from build123d import *

# Parameters (mm, degrees)
SKETCH1_W           = 480
SKETCH1_H           = 600
BOSS_EXTRUDE1_DEPTH = 40
SKETCH4_W           = 120
SKETCH4_H           = 440
CUT_EXTRUDE3_DEPTH  = 387.264158317
FILLET1_R           = 20
M24_TAPPED_HOLE1_D  = 21


with BuildPart() as part:
    # Sketch1 → Boss-Extrude1 (new body)
    with BuildSketch(Plane(origin=(0, 0, 0), x_dir=(1, 0, 0), z_dir=(0, 1, 0))):
        Rectangle(SKETCH1_W, SKETCH1_H)
    extrude(amount=BOSS_EXTRUDE1_DEPTH)

    # Sketch4 → Cut-Extrude3 (cut, through all)
    with BuildSketch(Plane(origin=(0, 40, 0), x_dir=(1, 0, 0), z_dir=(0, 1, 0))):
        with Locations((-112, 0)):
            Rectangle(SKETCH4_W, SKETCH4_H)
    extrude(amount=-CUT_EXTRUDE3_DEPTH, mode=Mode.SUBTRACT)

    # Fillet1
    fillet1_edges = [part.edges().sort_by_distance(p)[0] for p in [
        (-52, 20, -220),
        (-52, 20, 220),
        (-172, 20, 220),
        (-172, 20, -220),
    ]]
    fillet(fillet1_edges, radius=FILLET1_R)

    # M24 Tapped Hole1 (through all)
    with Locations(Plane(origin=(0, 40, 0), x_dir=(1, 0, 0), z_dir=(0, 1, 0))):
        with Locations((-190, -270), (-190, 270), (190, 270), (190, -270), (190, 170), (190, -170)):
            Hole(M24_TAPPED_HOLE1_D / 2)


solid = part.part
Geometry: final body of the model. Coordinates: model frame, mm. A direction names the side the tool comes from. Give positions to 0.01 mm unless a question says otherwise; leave off trailing zeros. Loops run counter-clockwise (first coordinate to the right, second up) from the corner with the lowest first, then second, coordinate; pieces in that order, holes last. Notation, with made-up numbers: (58.25, 83.25) - (73.25, 83.25) arc R12 ccw to (73.25, 103.25) - close; hole circle Ø6 at (-6, 55.5). An arc over 180 degrees is marked (long way). One line per question, with ' | ' between items. Start each with the question number.
(1) Contact query for a flat-ended pin moving along its axis: pin 1 (19 mm diameter, centred on x = 190, z = 170, fed in from +Y). Output: stop coordinate, or through.
(2) Ray query, line 1 (Z direction, x = 190, y = 17); line 2 (X direction, y = 13, z = 168.5); line 3 (X direction, y = 26, z = 270). Return the intervals inside material, ascending. Write a range as from..to.
(3) Section query C-C on z = -126.5. Return loops of the section in (x, y), then the cut area to 3 significant figures.
(4) Reachability of faces 4 (the flat face through (50, 0, -4)), 5 (the flat face through (-113, 20, 220)) from +Z, -Z, +X, -X, +Y, -Y: full face, straight path, thin tool, end or side. Return the list, or none.
(5) Section query B-B on x = -92.5. Return loops of the section in (y, z), then the cut area to 3 significant figures.
(6) Section query A-A on z = 170. Return loops of the section in (x, y).
(7) Pull-direction query (Z, two-part tool) for faces 1 (the flat face through (-52, 20, 3)), 2 (the flat face through (-3, 20, -300)), 3 (the flat face through (240, 20, 4)); classes: released by +Z, released by -Z, zero draft, split by the parting line, or undercut.
(8) Section query D-D on x = -190. Return loops of the section in (y, z).
The answers:
1) pin 1: through
2) line 1: -300..-280.5, -259.5..-180.5, -159.5..159.5, 180.5..259.5, 280.5..300 | line 2: -240..-172, -52..179.61, 200.39..240 | line 3: -240..-200.5, -179.5..179.5, 200.5..240
3) outline: (-240, 0) - (-172, 0) - (-172, 40) - (-240, 40) - close; (-52, 0) - (240, 0) - (240, 40) - (-52, 40) - close | area: 14,400 mm2
4) face 4: +Z, -Z, +X, -X, -Y | face 5: +Y, -Y
5) outline: (0, -300) - (40, -300) - (40, -220) - (0, -220) - close; (0, 220) - (40, 220) - (40, 300) - (0, 300) - close | area: 6,400 mm2
6) outline: (-240, 0) - (-172, 0) - (-172, 40) - (-240, 40) - close; (-52, 0) - (179.5, 0) - (179.5, 40) - (-52, 40) - close; (200.5, 0) - (240, 0) - (240, 40) - (200.5, 40) - close
7) face 1: undercut | face 2: released by -Z | face 3: zero draft
8) outline: (0, -300) - (40, -300) - (40, -280.5) - (0, -280.5) - close; (0, -259.5) - (40, -259.5) - (40, 259.5) - (0, 259.5) - close; (0, 280.5) - (40, 280.5) - (40, 300) - (0, 300) - close
